from build123d import *

# Parameters (mm, degrees)
SKETCH2_R           = 7
BOSS_EXTRUDE1_DEPTH = 10


with BuildPart() as part:
    # Sketch2 → Boss-Extrude1 (new body)
    with BuildSketch(Plane(origin=(0, 0, 0), x_dir=(1, 0, 0), z_dir=(0, 1, 0))):
        with BuildLine():
            Line((85, -20), (-85, -20))
            ThreePointArc((-85, -20), (-88.535533906, -18.535533906), (-90, -15))
            Line((-90, -15), (-90, 15))
            ThreePointArc((-90, 15), (-88.535533906, 18.535533906), (-85, 20))
            Line((-85, 20), (85, 20))
            ThreePointArc((85, 20), (88.535533906, 18.535533906), (90, 15))
            Line((90, 15), (90, -15))
            ThreePointArc((90, -15), (88.535533906, -18.535533906), (85, -20))
        make_face()
        with Locations(Location((-75, 0, 0), (0, 0, 270))):
            Circle(SKETCH2_R, mode=Mode.SUBTRACT)
        with Locations(Location((75, 0, 0), (0, 0, 90))):
            Circle(SKETCH2_R, mode=Mode.SUBTRACT)
    extrude(amount=BOSS_EXTRUDE1_DEPTH)


solid = part.part
Input: part model. Units: mm. Frame: model coordinates. Give positions to 0.01 mm unless a question says otherwise; leave off trailing zeros. Order: outer loops, then holes, each group sorted by start corner. A loop starts at its lowest first (then second) coordinate and runs counter-clockwise, first axis right, second up.
Q1. Ray query, probe 1 along X at (y, z) = (3, 0); probe 2 along X at (y, z) = (6.5, 1); probe 3 along Z at (x, y) = (75, 5.5). Return the intervals inside material, ascending.
Checked values:
probe 1: x = -90 to -82, -68 to 68, 82 to 90
probe 2: x = -90 to -81.93, -68.07 to 68.07, 81.93 to 90
probe 3: z = -20 to -7, 7 to 20
Q2. Section B-B on y = 4.5. Output: boundary loops of the cut face in (x, z).
Checked values:
outline: (-90, -15) arc R5 ccw to (-85, -20) - (85, -20) arc R5 ccw to (90, -15) - (90, 15) arc R5 ccw to (85, 20) - (-85, 20) arc R5 ccw to (-90, 15) - close; hole circle Ø14 at (-75, 0); hole circle Ø14 at (75, 0)
Q3. Section C-C on z = 0. Output: boundary loops of the cut face in (x, y), and give its area (3 significant figures).
Checked values:
outline: (-90, 0) - (-82, 0) - (-82, 10) - (-90, 10) - close; (-68, 0) - (68, 0) - (68, 10) - (-68, 10) - close; (82, 0) - (90, 0) - (90, 10) - (82, 10) - close
area: 1,520 mm2
Q4. Section A-A on x = -75. Output: boundary loops of the cut face in (y, z), and give its area (3 significant figures).
Checked values:
outline: (0, -20) - (10, -20) - (10, -7) - (0, -7) - close; (0, 7) - (10, 7) - (10, 20) - (0, 20) - close
area: 260 mm2
Q5. Draft query along Z for faces 1 (the flat face through (90, 5, 0)), 2 (the cylindrical face through (-68.06, 4.93, -0.91)), 3 (the cylindrical face through (-89, 5, -18)). Return one class per face: +Z half, -Z half, draft (parallel to the pull), parting line (faces both ways), or undercut.
Checked values:
face 1: draft
face 2: undercut
face 3: -Z half
